Work out the finished part from the listing and answer in its coordinate system (mm). Face numbers are marked on the shaded views. A direction names the side the tool comes from. Coordinates: 2 decimals unless noted, no trailing zeros. Write each loop counter-clockwise with the first axis right and the second up, starting at its lowest first coordinate (ties: lowest second). Pieces come first, ordered by that corner, then holes. Notation, with made-up numbers: (-23.5, -35) - (23.5, -35) arc R29 cw to (23.5, -5) - close; hole circle Ø2 at (72, 77). An arc over 180 degrees is marked (long way). Use a Markdown table: item, result. Add a question column.
(1) Given pin 1 Ø6 at (x, y) = (628, 365) entering from +Z; pin 2 Ø25 at (x, z) = (604.5, 114) entering from -Y; pin 3 Ø1 at (x, y) = (293.5, 98.5) entering from +Z, each flat-ended and moving along its own axis, determine where each tip first touches the part or whether it passes through.
(2) The part is cut by section B-B, the plane x = 407.5. Give the vertices of the cut face in (y, z).
(3) The part is cut by section A-A, the plane y = 33.5. Give the vertices of the cut face in (x, z).
(4) A tool of negligible diameter and unlimited length cuts with its end or side. For the marked faces 4, 5, 6 and 7, from which of +Z, -Z, +X, -X, +Y, -Y can it reach the whole face along a straight path? Write none if from no direction.
(5) For a pull along X with two mould halves and no side action, classify the marked faces 1, 2 and 3 as released by +X, released by -X, zero draft, split by the parting line, or undercut.
(6) The part is cut by section D-D, the plane x = 196.5. Give the vertices of the cut face in (y, z), then the cut area to 3 significant figures.
(7) Find the intervals of material crossed by line 1 (X direction, y = 240.5, z = 262); line 2 (X direction, y = 102, z = 156); line 3 (Z direction, x = 500.5, y = 226), in increasing order. Write a range as from..to.
(8) The part is cut by section C-C, the plane z = 81. Give the vertices of the cut face in (x, y).
from build123d import *

# Parameters (mm, degrees)
BASE_BLOCK_PROFILE_W            = 1000
BASE_BLOCK_PROFILE_H            = 540
BASE_BLOCK_DEPTH                = 200
RAISED_BLOCK_PROFILE_W          = 600
RAISED_BLOCK_PROFILE_H          = 300
RAISED_BLOCK_DEPTH              = 1000
RAISED_BLOCK_STEP_CUT_PROFILE_W = 1000
RAISED_BLOCK_STEP_CUT_PROFILE_H = 300
RAISED_BLOCK_STEP_CUT_DEPTH     = 100
STAIR_STEP_BOSS_PROFILE_W       = 200
STAIR_STEP_BOSS_PROFILE_H       = 100
STAIR_STEP_BOSS_DEPTH           = 150
STAIR_CUTOUT_DEPTH              = 150
STEPPED_SLOT_PROFILE_W          = 250
STEPPED_SLOT_PROFILE_H          = 80
STEPPED_SLOT_CUT_DEPTH          = 150
SLOT_SECOND_STEP_PROFILE_W      = 500
SLOT_SECOND_STEP_PROFILE_H      = 80
SLOT_SECOND_STEP_CUT_DEPTH      = 100
SLOT_THIRD_STEP_PROFILE_W       = 500
SLOT_THIRD_STEP_PROFILE_H       = 80
SLOT_THIRD_STEP_CUT_DEPTH       = 50


with BuildPart() as part:
    # Base Block Profile → Base Block (new body)
    with BuildSketch(Plane.XY):
        with Locations((500, 270)):
            Rectangle(BASE_BLOCK_PROFILE_W, BASE_BLOCK_PROFILE_H)
    extrude(amount=BASE_BLOCK_DEPTH)

    # Raised Block Profile → Raised Block (add)
    with BuildSketch(Plane(origin=(1000, 0, 0), x_dir=(0, 0, -1), z_dir=(1, 0, 0))):
        with Locations((-500, 390)):
            Rectangle(RAISED_BLOCK_PROFILE_W, RAISED_BLOCK_PROFILE_H)
    extrude(amount=-RAISED_BLOCK_DEPTH)

    # Raised Block Step Cut Profile → Raised Block Step Cut (cut)
    with BuildSketch(Plane.XY.offset(800)):
        with Locations((500, 390)):
            Rectangle(RAISED_BLOCK_STEP_CUT_PROFILE_W, RAISED_BLOCK_STEP_CUT_PROFILE_H)
    extrude(amount=-RAISED_BLOCK_STEP_CUT_DEPTH, mode=Mode.SUBTRACT)

    # Stair Step Boss Profile → Stair Step Boss (add)
    with BuildSketch(Plane(origin=(0, 540, 0), x_dir=(1, 0, 0), z_dir=(0, 1, 0))):
        with Locations((400, -750)):
            Rectangle(STAIR_STEP_BOSS_PROFILE_W, STAIR_STEP_BOSS_PROFILE_H)
        with Locations((600, -750)):
            Rectangle(STAIR_STEP_BOSS_PROFILE_W, STAIR_STEP_BOSS_PROFILE_H)
    extrude(amount=-STAIR_STEP_BOSS_DEPTH)

    # Stair Cutout Profile → Stair Cutout (cut)
    with BuildSketch(Plane.XZ.offset(-240)):
        Polygon((500, 700), (150, 700), (150, 200), (850, 200), (850, 700), align=None)
    extrude(amount=-STAIR_CUTOUT_DEPTH, mode=Mode.SUBTRACT)

    # Stepped Slot Profile → Stepped Slot Cut (cut)
    with BuildSketch(Plane.XY.offset(200)):
        with Locations((375, 40)):
            Rectangle(STEPPED_SLOT_PROFILE_W, STEPPED_SLOT_PROFILE_H)
        with Locations((625, 40)):
            Rectangle(STEPPED_SLOT_PROFILE_W, STEPPED_SLOT_PROFILE_H)
    extrude(amount=-STEPPED_SLOT_CUT_DEPTH, mode=Mode.SUBTRACT)

    # Slot Second Step Profile → Slot Second Step Cut (cut)
    with BuildSketch(Plane.XY.offset(200)):
        with Locations((500, 120)):
            Rectangle(SLOT_SECOND_STEP_PROFILE_W, SLOT_SECOND_STEP_PROFILE_H)
    extrude(amount=-SLOT_SECOND_STEP_CUT_DEPTH, mode=Mode.SUBTRACT)

    # Slot Third Step Profile → Slot Third Step Cut (cut)
    with BuildSketch(Plane.XY.offset(200)):
        with Locations((500, 200)):
            Rectangle(SLOT_THIRD_STEP_PROFILE_W, SLOT_THIRD_STEP_PROFILE_H)
    extrude(amount=-SLOT_THIRD_STEP_CUT_DEPTH, mode=Mode.SUBTRACT)


solid = part.part
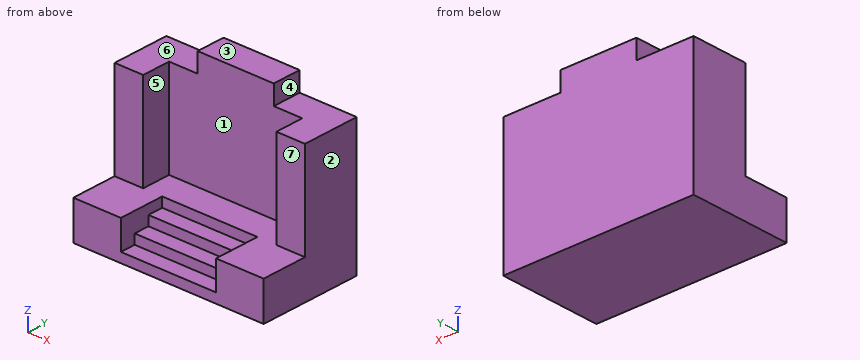
Model answer:
| question | item | result |
|---|---|---|
| 1 | pin 1 | z = 200 |
| 1 | pin 2 | y = 160 |
| 1 | pin 3 | z = 100 |
| 2 | outline | (0, 0) - (540, 0) - (540, 800) - (390, 800) - (390, 200) - (240, 200) - (240, 150) - (160, 150) - (160, 100) - (80, 100) - (80, 50) - (0, 50) - close |
| 3 | outline | (0, 0) - (1000, 0) - (1000, 200) - (750, 200) - (750, 50) - (250, 50) - (250, 200) - (0, 200) - close |
| 4 | face 4 | +Z, +X, +Y, -Y |
| 4 | face 5 | +Z, -Y |
| 4 | face 6 | +Z, -X, +Y, -Y |
| 4 | face 7 | +Z, +X, -X, -Y |
| 5 | face 1 | undercut |
| 5 | face 2 | released by +X |
| 5 | face 3 | zero draft |
| 6 | outline | (0, 0) - (540, 0) - (540, 700) - (390, 700) - (390, 200) - (0, 200) - close |
| 6 | area | 183,000 mm^2 |
| 7 | line 1 | 0..150, 850..1000 |
| 7 | line 2 | 0..250, 750..1000 |
| 7 | line 3 | 0..150 |
| 8 | outline | (0, 0) - (250, 0) - (250, 80) - (750, 80) - (750, 0) - (1000, 0) - (1000, 540) - (0, 540) - close |
